CAD build for the part. Positions are in the model's coordinates, mm. A direction names the side the tool comes from. Coordinates: 2 decimals unless noted, no trailing zeros. Order: outer loops, then holes, each group sorted by start corner. A loop starts at its lowest first (then second) coordinate and runs counter-clockwise, first axis right, second up. Notation, with made-up numbers: M 46,-28.75 L 86,-28.75 A5 cw 86,-23.75 Z; hole C 56,1.25 d3. An arc over 180 degrees is marked long. Write item = value, one per line.
from build123d import *

# Parameters (mm, degrees)
BASE_PLATE_SKETCH_R       = 5
BASE_PLATE_DEPTH          = 20
PLATE_HOLES_12_DEPTH      = 114.578166916
PLATE_HOLES_12_DEPTH_BACK = 114.578166916
PLATE_HOLES_SKETCH_W      = 25
PLATE_HOLES_SKETCH_H      = 12
SQUARE_BOSS_DEPTH         = 50
BOSS_HOLE_16_DEPTH        = 125.295950858
BOSS_HOLE_16_DEPTH_BACK   = 125.295950858
BOSS_HOLE_SKETCH_R        = 8
BOSS_CHAMFER_25X45_SIZE   = 25
SLOT_CUT_DEPTH            = 122.4197622
SLOT_CUT_DEPTH_BACK       = 122.4197622


with BuildPart() as part:
    # Base Plate Sketch → Base Plate (new body)
    with BuildSketch(Plane.XY):
        with BuildLine():
            Line((-35, 50), (35, 50))
            ThreePointArc((35, 50), (45.606601718, 45.606601718), (50, 35))
            Line((50, 35), (50, -35))
            ThreePointArc((50, -35), (45.606601718, -45.606601718), (35, -50))
            Line((35, -50), (-35, -50))
            ThreePointArc((-35, -50), (-45.606601718, -45.606601718), (-50, -35))
            Line((-50, -35), (-50, 35))
            ThreePointArc((-50, 35), (-45.606601718, 45.606601718), (-35, 50))
        make_face()
        with Locations((-35, 35)):
            Circle(BASE_PLATE_SKETCH_R, mode=Mode.SUBTRACT)
        with Locations((35, 35)):
            Circle(BASE_PLATE_SKETCH_R, mode=Mode.SUBTRACT)
        with Locations((35, -35)):
            Circle(BASE_PLATE_SKETCH_R, mode=Mode.SUBTRACT)
        with Locations((-35, -35)):
            Circle(BASE_PLATE_SKETCH_R, mode=Mode.SUBTRACT)
    extrude(amount=BASE_PLATE_DEPTH)

    # Plate Holes Sketch → Plate Holes Ø12 (cut, two sides: drawn at the far end of the back side and taken through both)
    with BuildSketch(Plane.XZ.offset(50).offset(-PLATE_HOLES_12_DEPTH_BACK)):
        Rectangle(PLATE_HOLES_SKETCH_W, PLATE_HOLES_SKETCH_H)
    extrude(amount=PLATE_HOLES_12_DEPTH + PLATE_HOLES_12_DEPTH_BACK, mode=Mode.SUBTRACT)

    # Square Boss Sketch → Square Boss (add)
    with BuildSketch(Plane.XY.offset(20)):
        Polygon((-42.779960262, 2.474873734), (-2.474873734, 42.779960262), (42.779960262, -2.474873734), (2.474873734, -42.779960262), align=None)
    extrude(amount=SQUARE_BOSS_DEPTH)

    # Boss Hole Sketch → Boss Hole Ø16 (cut, two sides: drawn at the far end of the back side and taken through both)
    with BuildSketch(Plane(origin=(22.627416998, -22.627416998, 0), x_dir=(0, 0, -1), z_dir=(0.7071067811865462, -0.7071067811865488, 0)).offset(-BOSS_HOLE_16_DEPTH_BACK)):
        with Locations(Location((-52, 3.5, 0), (0, 0, 90))):
            Circle(BOSS_HOLE_SKETCH_R)
    extrude(amount=BOSS_HOLE_16_DEPTH + BOSS_HOLE_16_DEPTH_BACK, mode=Mode.SUBTRACT)

    # Boss Chamfer 25x45°
    boss_chamfer_25x45_edges = [part.edges().sort_by_distance(p)[0] for p in [
        (-20.152543264, -20.152543264, 70),
    ]]
    chamfer(boss_chamfer_25x45_edges, length=BOSS_CHAMFER_25X45_SIZE)

    # Slot Sketch → Slot Cut (cut, two sides: drawn at the far end of the back side and taken through both)
    with BuildSketch(Plane(origin=(20.152543264, 20.152543264, 0), x_dir=(0, 0, -1), z_dir=(0.7071067811865486, 0.7071067811865465, 0)).offset(-SLOT_CUT_DEPTH_BACK)):
        Polygon((-70, 16), (-40, 16), (-26, 0), (-40, -16), (-70, -16), align=None)
    extrude(amount=SLOT_CUT_DEPTH + SLOT_CUT_DEPTH_BACK, mode=Mode.SUBTRACT)


solid = part.part
(1) Pull direction Y, two halves, no side cores. Call faces 1 (the face through (-15.311, 18.788, 59.932)), 2 (the face through (0, 1, 6)), 3 (the face through (-6.018, 5.454, 33.098)), 4 (the face through (-22.91, 22.345, 39.094)): +Y half, -Y half, draft (parallel to the pull), parting line (faces both ways), or undercut.
Evaluation:
face_1 = undercut
face_2 = draft
face_3 = undercut
face_4 = +Y half
(2) Wall check: line 1 (Y direction, x = 35, z = 4.75); line 2 (Z direction, x = 13, y = -33); line 3 (Z direction, x = -10.5, y = -35.5). Give the ranges that are in metal, low to high. Write a range as from..to.
Evaluation:
line_1 = -50..-40, -30..30, 40..50
line_2 = 0..20
line_3 = 6..20
(3) Slice it at A-A, the plane z = 16. Write the cut outline in (x, y), then the cut area to 3 significant figures.
Evaluation:
outline = M -50,-35 A15 ccw -35,-50 L 35,-50 A15 ccw 50,-35 L 50,35 A15 ccw 35,50 L -35,50 A15 ccw -50,35 Z; hole C -35,-35 d10; hole C -35,35 d10; hole C 35,-35 d10; hole C 35,35 d10
area = 9,490 mm²
(4) Slice it at B-B, the plane z = 30.5. Write the cut outline in (x, y), then the cut area to 3 significant figures.
Evaluation:
outline = M -42.78,2.47 L -23.79,-16.52 L 16.52,23.79 L -2.47,42.78 Z; M -16.52,-23.79 L 2.47,-42.78 L 42.78,-2.47 L 23.79,16.52 Z
area = 3,060 mm²
(5) Tool access for faces 5 (the face through (24.864, 15.441, 27.983)), 6 (the face through (23, 23, 20)), 7 (the face through (-19.836, -20.469, 23.992)), 8 (the face through (22.91, -22.345, 39.094)): list every direction of +Z, -Z, +X, -X, +Y, -Y with a clear straight run to the whole face (end or side of a thin tool).
Evaluation:
face_5 = +Z, +X, +Y
face_6 = +Z
face_7 = +Z, -X, -Y
face_8 = +Z, +X, -Y
(6) Pin check, flat tips, straight feed: pin 1 Ø2 at (x, y) = (7, 26) entering from -Z; pin 2 Ø5 at (y, z) = (-5, 60.5) entering from -X; pin 3 Ø13 at (x, y) = (35, -35) entering from +Z; pin 4 Ø9 at (x, y) = (35, 35) entering from -Z. Stop position of each tip, or through.
Evaluation:
pin_1 = 6
pin_2 = 15.13
pin_3 = 20
pin_4 = through
